The figure shows three views and two pictorial views of one solid part (mm, origin at its lowest corner). Answer the questions. A direction names the side the tool comes from. Give positions to 0.01 mm unless a question says otherwise; leave off trailing zeros. Order: outer loops, then holes, each group sorted by start corner. A loop starts at its lowest first (then second) coordinate and runs counter-clockwise, first axis right, second up. Notation, with made-up numbers: (88.5, 51) - (101.5, 51) arc R16 cw to (101.5, 65) - close; hole circle Ø9 at (-18.75, 79.25). An arc over 180 degrees is marked (long way). Answer as CSV lines item,"result". Start each with the question number.
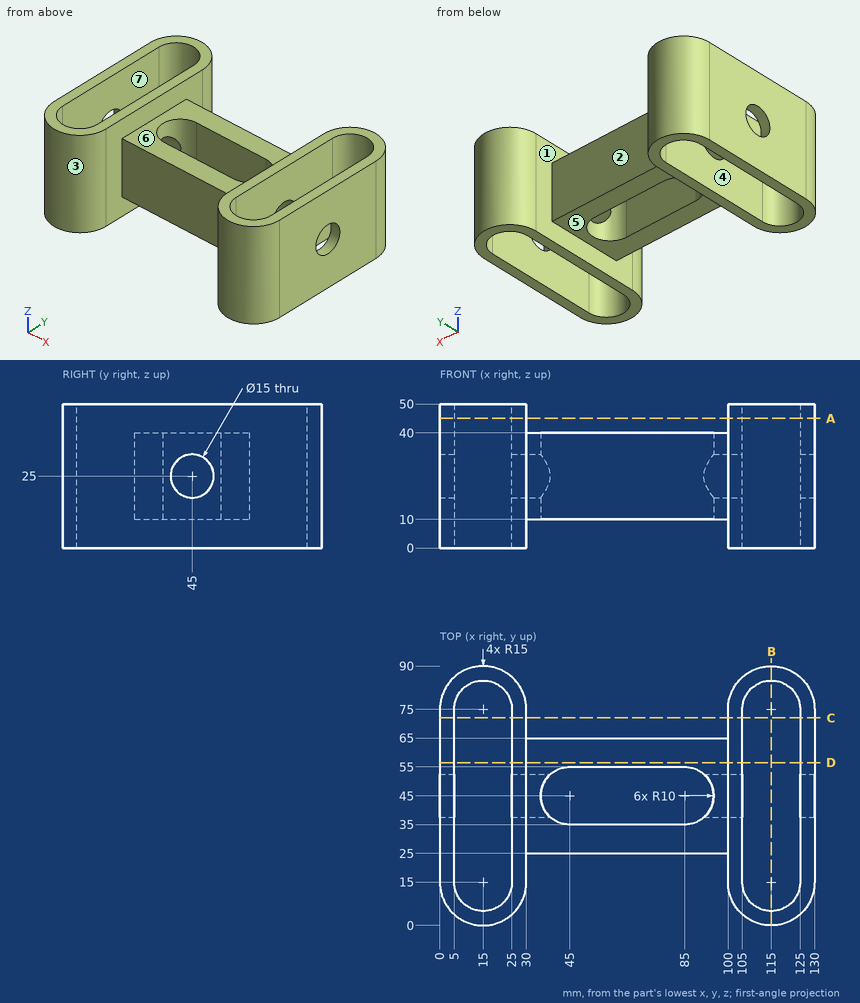
(1) Straight lines are drawn through the part: line 1 (X direction, y = 62.5, z = 26.5); line 2 (X direction, y = 23.5, z = 10.5); line 3 (Z direction, x = 97, y = 45). For each, find the intervals that lie inside material, in ascending order. Write a range as [from, to].
(2) Section A-A, the plane z = 45 is taken. Write down the section's boundary in (x, y), and give its area (3 significant figures).
(3) Determine the mould class of the marked faces 1, 2, 3 and 4 for opening direction Y: released by +Y, released by -Y, zero draft, split by the parting line, or undercut.
(4) Section C-C, the plane y = 72 is taken. Write down the section's boundary in (x, z), and give its area (3 significant figures).
(5) Section D-D, the plane y = 56.5 is taken. Write down the section's boundary in (x, z), and give its area (3 significant figures).
(6) Flat-ended cylindrical pins translate along their axes: pin 1 Ø13.5 at (y, z) = (45, 25) entering from +X (3 decimals); pin 2 Ø6 at (x, z) = (110.5, 19) entering from -Y; pin 3 Ø3 at (y, z) = (20, 8.5) entering from -X; pin 4 Ø15 at (x, z) = (76.5, 21.5) entering from +Y. Find the tip coordinate at first contact, or state that the pin passes through.
(7) Which of the six approach directions +Z, -Z, +X, -X, +Y, -Y give full straight-line access (tool end or side, diameter ignored) to the marked faces 5, 6 and 7?
(8) Section B-B, the plane x = 115 is taken. Write down the section's boundary in (y, z), and give its area (3 significant figures).
Checks:
1,line 1,"x = [0, 5], [25, 105], [125, 130]"
1,line 2,"x = [0, 5], [25, 30], [100, 105], [125, 130]"
1,line 3,"z = [10, 17.5], [32.5, 40]"
2,outline,"(0, 15) arc R15 ccw to (30, 15) - (30, 75) arc R15 ccw to (0, 75) - close; (100, 15) arc R15 ccw to (130, 15) - (130, 75) arc R15 ccw to (100, 75) - close; hole (5, 15) arc R10 ccw to (25, 15) - (25, 75) arc R10 ccw to (5, 75) - close; hole (105, 15) arc R10 ccw to (125, 15) - (125, 75) arc R10 ccw to (105, 75) - close"
2,area,"1,990 mm²"
3,face 1,"zero draft"
3,face 2,"released by +Y"
3,face 3,"released by -Y"
3,face 4,"undercut"
4,outline,"(0, 0) - (5, 0) - (5, 50) - (0, 50) - close; (25, 0) - (30, 0) - (30, 50) - (25, 50) - close; (100, 0) - (105, 0) - (105, 50) - (100, 50) - close; (125, 0) - (130, 0) - (130, 50) - (125, 50) - close"
4,area,"1,000 mm²"
5,outline,"(0, 0) - (5, 0) - (5, 50) - (0, 50) - close; (25, 0) - (30, 0) - (30, 10) - (100, 10) - (100, 0) - (105, 0) - (105, 50) - (100, 50) - (100, 40) - (30, 40) - (30, 50) - (25, 50) - close; (125, 0) - (130, 0) - (130, 50) - (125, 50) - close"
5,area,"3,100 mm²"
6,pin 1,"passes through"
6,pin 2,"stops at y = 0.08"
6,pin 3,"stops at x = 0"
6,pin 4,"stops at y = 65"
7,face 5,"-Z, +Y, -Y"
7,face 6,"+Z, +Y, -Y"
7,face 7,"+Z, -Z"
8,outline,"(0, 0) - (5, 0) - (5, 50) - (0, 50) - close; (85, 0) - (90, 0) - (90, 50) - (85, 50) - close"
8,area,"500 mm²"
